Model file for the job. Use its own axes, mm. A direction names the side the tool comes from. Coordinates: 2 decimals unless noted, no trailing zeros. Order: outer loops, then holes, each group sorted by start corner. A loop starts at its lowest first (then second) coordinate and runs counter-clockwise, first axis right, second up. Notation, with made-up numbers: (16, -20) -> (45, -20) arc R19 ccw to (45, -6) -> close; hole circle Ø2 at (45, 4). An arc over 180 degrees is marked (long way). Write item = value, one per line. Start each with the question number.
Q1. Cut at A-A, the plane y = -25. List the corners of the cut face in (x, z).
Q2. Flat gauge pin, fed straight in: pin 1 (1 mm diameter, centred on x = 31, z = 91.5, fed in from -Y). Where does the tip first touch, or does it go through?
Q3. Mould opens along X. For faces 1 (the face through (50.2, -4.5, 0)), 2 (the face through (0, -25, 86)), 3 (the face through (5, -27, 86)) say: +X half, -X half, draft (parallel to the pull), parting line (faces both ways), or undercut.
Q4. Wall check: line 1 (X direction, y = -7.5, z = 79); line 2 (Y direction, x = 73, z = 119.5). Give the ranges that are in metal, low to high. Write a range as from..to.
Q5. 3-axis set-ups, long thin cutter, end or side, ignore diameter. For faces 4 (the face through (50.2, -4.5, 175)), 5 (the face through (95, -28, 86)): which of +Z, -Z, +X, -X, +Y, -Y reach the whole face in a straight line?
Q6. Cut at B-B, the plane z = 81. List the corners of the cut face in (x, y), plus the area to 3 significant figures.
Q7. Cut at C-C, the plane x = 33. List the corners of the cut face in (y, z), plus the area to 3 significant figures.
from build123d import *

# Parameters (mm, degrees)
EXTRUDE_1_DEPTH = 175


with BuildPart() as part:
    # 草图1 → 凸台-拉伸1 (new body)
    with BuildSketch(Plane.XY):
        Polygon((0, 0), (100, 0), (100, -50), (95, -50), (95, -5), (5, -5), (5, -50), (0, -50), align=None)
    extrude(amount=EXTRUDE_1_DEPTH)


solid = part.part
Here are the results:
q1.outline = (0, 0) -> (5, 0) -> (5, 175) -> (0, 175) -> close; (95, 0) -> (100, 0) -> (100, 175) -> (95, 175) -> close
q2.pin_1 = -5
q3.face_1 = draft
q3.face_2 = -X half
q3.face_3 = undercut
q4.line_1 = 0..5, 95..100
q4.line_2 = -5..0
q5.face_4 = +Z, +X, -X, +Y, -Y
q5.face_5 = +Z, -Z, -Y
q6.outline = (0, -50) -> (5, -50) -> (5, -5) -> (95, -5) -> (95, -50) -> (100, -50) -> (100, 0) -> (0, 0) -> close
q6.area = 950 mm²
q7.outline = (-5, 0) -> (0, 0) -> (0, 175) -> (-5, 175) -> close
q7.area = 875 mm²
